The model under review builds one solid part; all positions refer to its coordinate system, in mm. Face numbers are marked on the shaded views. A direction names the side the tool comes from. Round coordinates to 2 decimals unless told otherwise and drop trailing zeros. Write each loop counter-clockwise with the first axis right and the second up, starting at its lowest first coordinate (ties: lowest second). Pieces come first, ordered by that corner, then holes. Notation, with made-up numbers: (56, 35) -> (114, 35) arc R16 ccw to (114, 42) -> close; hole circle Ø1 at (-11, 15.5). An arc over 180 degrees is marked (long way). Answer as a JSON object with one key per item and string values. Group by question number.
1) To check wall thickness, follow probe 1 along X at (y, z) = (12, -15); probe 2 along Z at (x, y) = (15.5, 0.5); probe 3 along X at (y, z) = (12, 10) (3 decimals). State the ranges of each line that lie inside material, in increasing order. Write a range as [from, to].
2) Mouldability with a two-part tool opening along X and no side actions: class the marked faces 6, 7 and 8 as pulls with the +X half, pulls with the -X half, needs draft (parallel to the pull), parting line crosses it, or undercut.
3) We need section A-A, the plane x = 6. Write out the cut boundary in (y, z), then the cut area to 3 significant figures.
4) We need section B-B, the plane x = 13. Write out the cut boundary in (y, z), then the cut area to 3 significant figures.
5) We need section C-C, the plane x = 28. Write out the cut boundary in (y, z).
6) Machinability: for the marked faces 1, 2, 3, 4 and 5, which of the approach directions +Z, -Z, +X, -X, +Y, -Y give a long, thin tool a straight path to every point of the face, cutting with its end or side? Answer none if there is none.
7) Insertion check: pin 1 Ø10 at (x, z) = (17.5, -2) entering from -Y; pin 2 Ø8 at (x, y) = (11.5, -5) entering from +Z; pin 3 Ø3.5 at (x, y) = (4, 3.5) entering from -Z. Each pin has a flat end and moves straight along its axis. Give the tip position at first contact, or say it passes through.
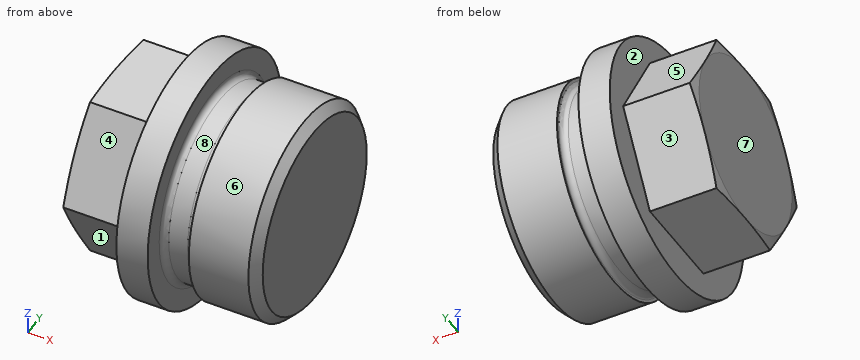
from build123d import *

# Parameters (mm, degrees)
EXTRUDE1_DEPTH     = 11
SKETCH3_OUTSIDE_W  = 167.178
SKETCH3_OUTSIDE_H  = 167.178
SKETCH3_OUTSIDE_R  = 13.5
CUT_EXTRUDE1_DEPTH = 10
CUT_EXTRUDE1_DRAFT = -80
FILLET1_R          = 1


with BuildPart() as part:
    # Sketch1 → Revolve1 (revolve)
    with BuildSketch(Plane.XY, mode=Mode.PRIVATE) as revolve1_sk:
        Polygon((21, 16.6245), (21, 15.1455), (16, 15.1455), (16, 19.5), (11, 19.5), (11, 1.5), (0, 1.5), (0, 0), (32, 0), (32, 15.1455), (30.521, 16.6245), align=None)
    revolve(revolve1_sk.sketch.rotate(Axis((0, 0, 0), (1, 0, 0)), 90), axis=Axis((0, 0, 0), (1, 0, 0)))

    # Sketch2 → Extrude1 (add)
    with BuildSketch(Plane.ZY):
        Polygon((0, 15.588457268), (-13.5, 7.794228634), (-13.5, -7.794228634), (0, -15.588457268), (13.5, -7.794228634), (13.5, 7.794228634), align=None)
    extrude(amount=-EXTRUDE1_DEPTH)


with BuildPart() as cut_extrude1_tool:
    # Sketch3 outside → Cut-Extrude1 (with draft: the straight prism first)
    with BuildSketch(Plane.ZY):
        Rectangle(SKETCH3_OUTSIDE_W, SKETCH3_OUTSIDE_H)
        Circle(SKETCH3_OUTSIDE_R, mode=Mode.SUBTRACT)
    extrude(amount=-CUT_EXTRUDE1_DEPTH)
    # Cut-Extrude1: the draft: its side faces are tilted about the plane it starts from
    cut_extrude1_sides = [cut_extrude1_tool.faces().sort_by_distance(p)[0] for p in [
        (5, -83.589, 0),
        (5, 0, 83.589),
        (5, 83.589, 0),
        (5, 0, -83.589),
        (5, 0, -13.5),
    ]]
    draft(cut_extrude1_sides, Plane.ZY, CUT_EXTRUDE1_DRAFT)


with BuildPart() as part_1:
    add(part.part)

    # Cut-Extrude1: cut by cut_extrude1_tool
    add(cut_extrude1_tool.part, mode=Mode.SUBTRACT)

    # Fillet1
    fillet1_edges = [part_1.edges().sort_by_distance(p)[0] for p in [
        (21, 0, -15.1455),
        (16, 0, -15.1455),
    ]]
    fillet(fillet1_edges, radius=FILLET1_R)


solid = part_1.part
Here are the results:
{
 "1": {"probe 1": "x = [11, 16]", "probe 2": "z = [-19.49, 19.49]", "probe 3": "x = [11, 16.149], [20.851, 31.525]"},
 "2": {"face 6": "needs draft", "face 7": "pulls with the -X half", "face 8": "undercut"},
 "3": {"outline": "(-15.59, 0) -> (-7.79, -13.5) -> (7.79, -13.5) -> (15.59, 0) -> (7.79, 13.5) -> (-7.79, 13.5) -> close", "area": "631 mm^2"},
 "4": {"outline": "circle Ø39 at (0, 0)", "area": "1,190 mm^2"},
 "5": {"outline": "circle Ø33.25 at (0, 0)"},
 "6": {"face 1": "-Z, -X, -Y", "face 2": "-X", "face 3": "-Z, -X, +Y", "face 4": "+Z, -X, -Y", "face 5": "+Z, -X, +Y"},
 "7": {"pin 1": "stops at y = -19.5", "pin 2": "stops at z = 19.47", "pin 3": "stops at z = -13.5"}
}
